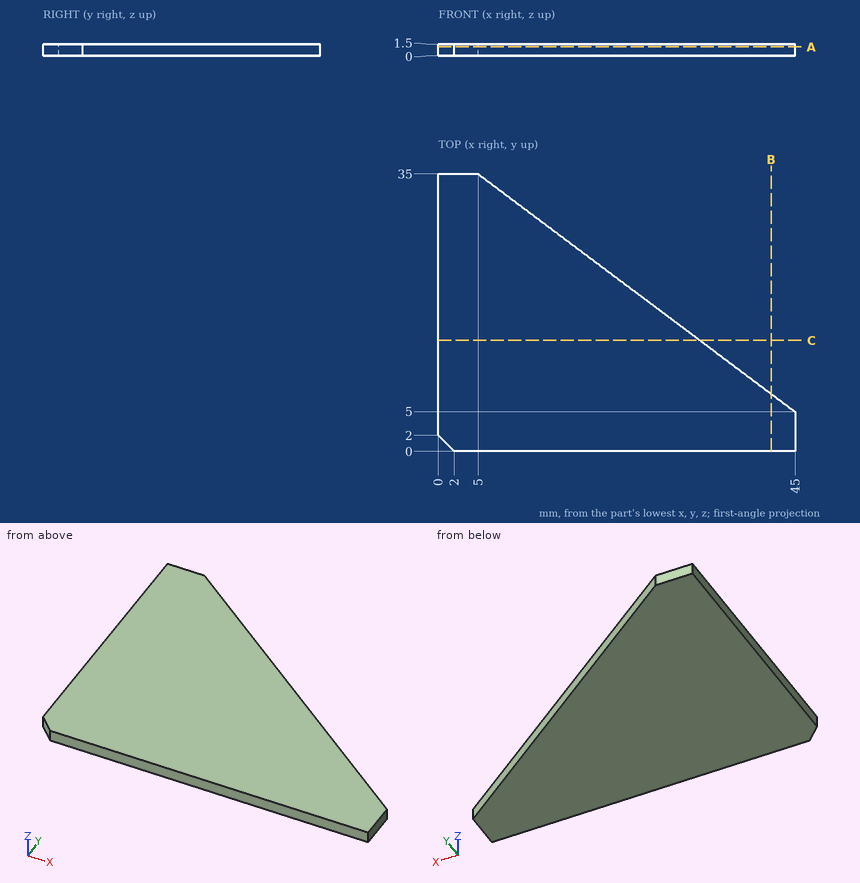
Part print with two shaded views. Sizes in mm from the minimum x, y, z corner. Coordinates: 2 decimals unless noted, no trailing zeros. Write each loop counter-clockwise with the first axis right and the second up, starting at its lowest first coordinate (ties: lowest second). Pieces come first, ordered by that corner, then holes. Notation, with made-up numbers: (-12, 32) - (47, 32) arc R20 cw to (47, 66) - close; hole circle Ø2 at (-19, -10). An arc over 180 degrees is marked (long way). Use a Markdown table: item, result. Add a question column.
Item 1: Band-saw the part on B-B, the plane x = 42. Write the cut outline in (y, z), and give its area (3 significant figures).
Item 2: Band-saw the part on C-C, the plane y = 14. Write the cut outline in (x, z).
Item 3: Drill centre lines: line 1 along X through (y, z) = (7, 1.4); line 2 along X through (y, z) = (26, 0.85); line 3 along Y through (x, z) = (39, 1.15). Where is each one in solid material? Low to high.
Item 4: Band-saw the part on A-A, the plane z = 1.15. Write the cut outline in (x, y), and give its area (3 significant figures).
A:
| question | item | result |
|---|---|---|
| 1 | outline | (0, 0) - (7.25, 0) - (7.25, 1.5) - (0, 1.5) - close |
| 1 | area | 10.9 mm² |
| 2 | outline | (0, 0) - (33, 0) - (33, 1.5) - (0, 1.5) - close |
| 3 | line 1 | x = 0 to 42.33 |
| 3 | line 2 | x = 0 to 17 |
| 3 | line 3 | y = 0 to 9.5 |
| 4 | outline | (0, 2) - (2, 0) - (45, 0) - (45, 5) - (5, 35) - (0, 35) - close |
| 4 | area | 973 mm² |
